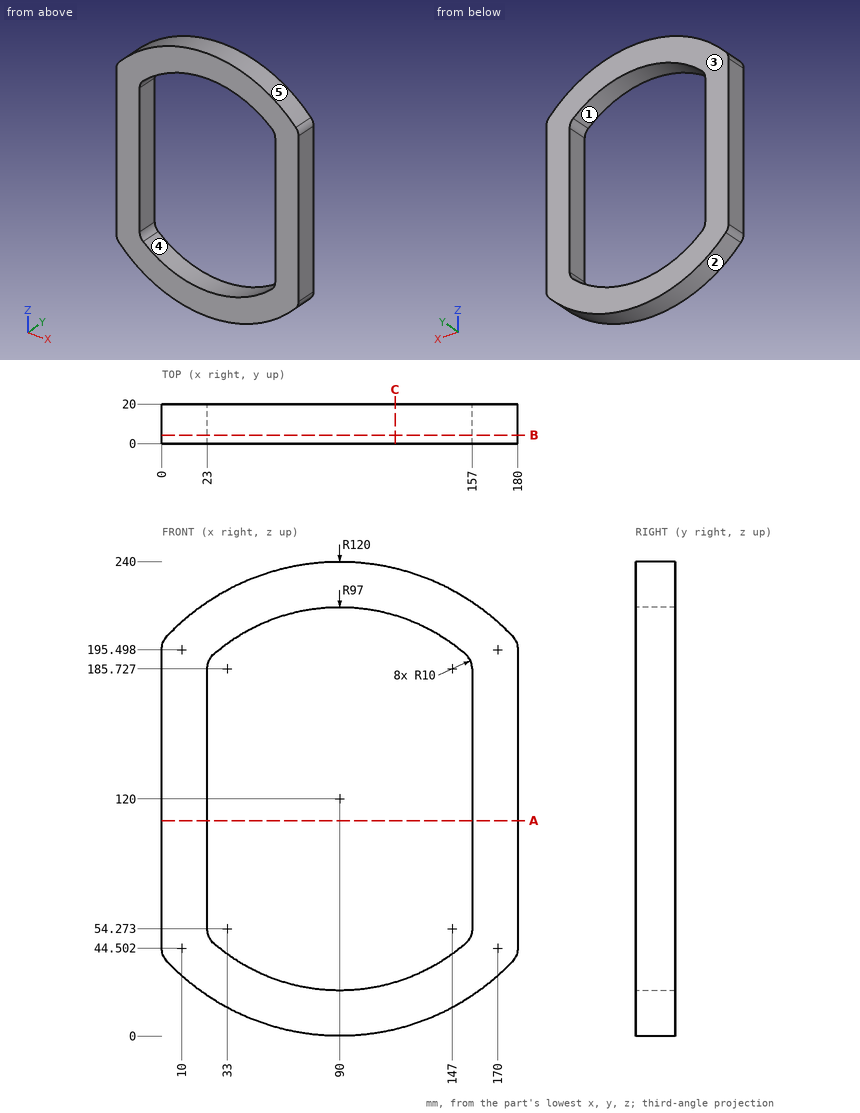
The figure shows three views and two pictorial views of one solid part (mm, origin at its lowest corner). Answer the questions. A direction names the side the tool comes from. Round coordinates to 2 decimals unless told otherwise and drop trailing zeros. Order: outer loops, then holes, each group sorted by start corner. A loop starts at its lowest first (then second) coordinate and runs counter-clockwise, first axis right, second up. Notation, with made-up numbers: (-9, 22.5) -> (20, 22.5) arc R27 ccw to (20, 54.5) -> close; hole circle Ø7 at (40.25, 57.25). An arc over 180 degrees is marked (long way). Put each result on its own line as item: value.
Q1. Section A-A, the plane z = 109 is taken. Write down the section's boundary in (x, y).
Results list:
outline: (0, 0) -> (23, 0) -> (23, 20) -> (0, 20) -> close; (157, 0) -> (180, 0) -> (180, 20) -> (157, 20) -> close
Q2. Determine the mould class of the marked faces 1, 2 and 3 for opening direction X: pulls with the +X half, pulls with the -X half, needs draft (parallel to the pull), parting line crosses it, or undercut.
Results list:
face 1: undercut
face 2: parting line crosses it
face 3: needs draft
Q3. Section B-B, the plane y = 4.25 is taken. Write down the section's boundary in (x, z), and give its area (3 significant figures).
Results list:
outline: (0, 44.5) arc R10 ccw to (2.73, 37.64) arc R120 ccw to (177.27, 37.64) arc R10 ccw to (180, 44.5) -> (180, 195.5) arc R10 ccw to (177.27, 202.36) arc R120 ccw to (2.73, 202.36) arc R10 ccw to (0, 195.5) -> close; hole (23, 54.27) arc R10 ccw to (26.45, 46.72) arc R97 ccw to (153.55, 46.72) arc R10 ccw to (157, 54.27) -> (157, 185.73) arc R10 ccw to (153.55, 193.28) arc R97 ccw to (26.45, 193.28) arc R10 ccw to (23, 185.73) -> close
area: 15,000 mm^2
Q4. Which of the six approach directions +Z, -Z, +X, -X, +Y, -Y give full straight-line access (tool end or side, diameter ignored) to the marked faces 4 and 5?
Results list:
face 4: +Y, -Y
face 5: +Z, +Y, -Y
Q5. Consider line 1 along X through (y, z) = (15, 178.5); line 2 along Z through (x, y) = (134, 7.25); line 3 along Z through (x, y) = (72, 9.75) (1 decimal). Determine where each line is inside the solid, lowest interval first.
Results list:
line 1: 0 to 23, 157 to 180
line 2: 8.36 to 33.55, 206.45 to 231.64
line 3: 1.4 to 24.7, 215.3 to 238.6
Q6. Each of these flat-tipped pins is pushed along its axis until it touches: P1, Ø10, axis at y = 10, z = 203, coming from the -X side; P2, Ø5, axis at x = 74.5, y = 16.5, coming from the -Z side; P3, Ø3, axis at y = 10, z = 33, coming from the -X side. Where does it stop, or does it pass through?
Results list:
P1: x = 0.32
P2: z = 0.71
P3: x = 5.8
Q7. Section C-C, the plane x = 118 is taken. Write down the section's boundary in (y, z).
Results list:
outline: (0, 3.31) -> (20, 3.31) -> (20, 27.13) -> (0, 27.13) -> close; (0, 212.87) -> (20, 212.87) -> (20, 236.69) -> (0, 236.69) -> close
